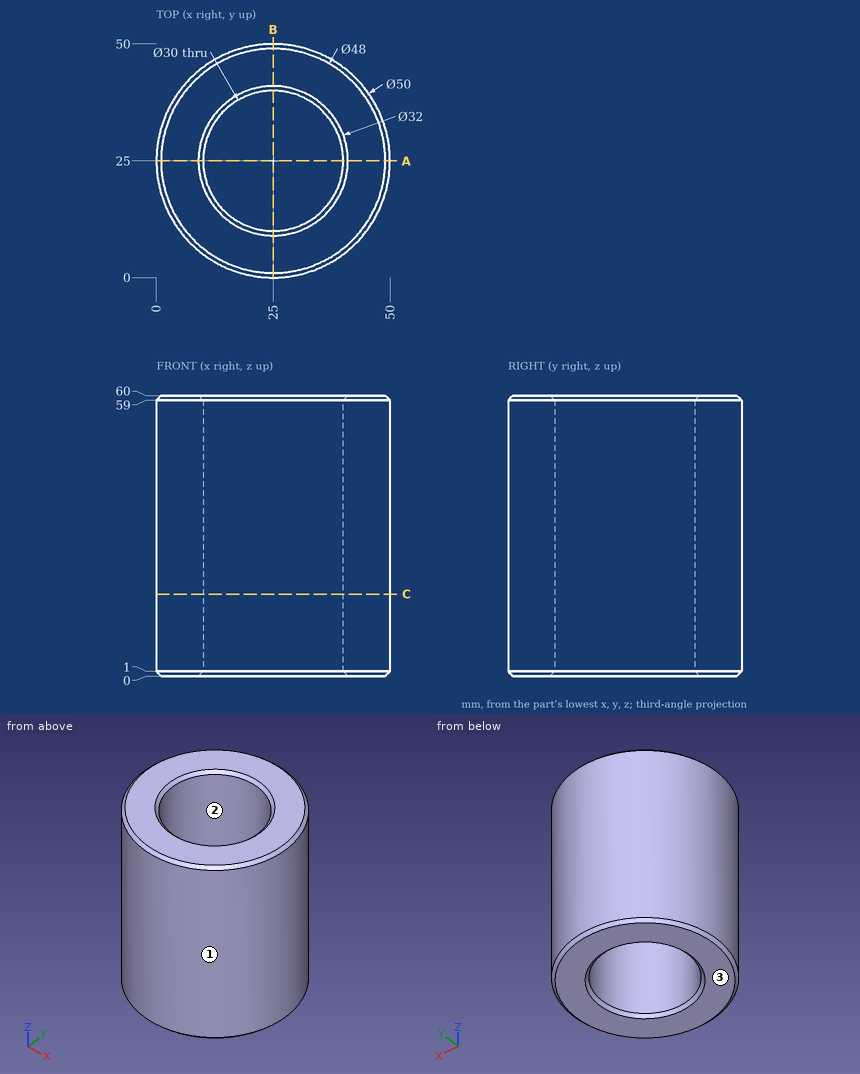
Here's the drawing with two shaded views (mm, measured from the low corner). I have some questions. Round coordinates to 2 decimals unless told otherwise and drop trailing zeros. Loops run counter-clockwise (first coordinate to the right, second up) from the corner with the lowest first, then second, coordinate; pieces in that order, holes last. Notation, with made-up numbers: M -9,5.5 L 23,5.5 A27 cw 23,36.5 Z; hole C 32,39 d8. An arc over 180 degrees is marked long. Answer as a JSON object with one key per item and string values. Group by question number.
Q1. We'd pull the mould along X, two halves only. Please class the marked faces 1, 2 and 3: +X half, -X half, draft (parallel to the pull), parting line (faces both ways), or undercut.
Q2. Imagine slicing it at A-A, the plane y = 25. Please give me the cut outline in (x, z), then the cut area to 3 significant figures.
Q3. Please list where these lines run through material, in increasing order: L1, parallel to Y at x = 25, z = 45.5; L2, parallel to Y at x = 19, z = 54; L3, parallel to X at y = 25.5, z = 20.5 (3 decimals).
Q4. Imagine slicing it at C-C, the plane z = 17.5. Please give me the cut outline in (x, y).
Q5. Will these pins go through, and if not, where does the flat tip stop? pin 1 (4 mm diameter, centred on y = 18, z = 34.5, fed in from -X); pin 2 (5 mm diameter, centred on x = 34.5, y = 38, fed in from -Z); pin 3 (5 mm diameter, centred on x = 26.5, y = 37, fed in from -Z); pin 4 (1.5 mm diameter, centred on x = 29.5, y = 11, fed in from -Z).
Findings:
{
 "1": {"face 1": "parting line", "face 2": "undercut", "face 3": "draft"},
 "2": {"outline": "M 0,1 L 1,0 L 9,0 L 10,1 L 10,59 L 9,60 L 1,60 L 0,59 Z; M 40,1 L 41,0 L 49,0 L 50,1 L 50,59 L 49,60 L 41,60 L 40,59 Z", "area": "1,200 mm2"},
 "3": {"L1": "y = 0 to 10, 40 to 50", "L2": "y = 0.73 to 11.25, 38.75 to 49.27", "L3": "x = 0.005 to 10.008, 39.992 to 49.995"},
 "4": {"outline": "C 25,25 d50; hole C 25,25 d30"},
 "5": {"pin 1": "stops at x = 0.51", "pin 2": "stops at z = 0", "pin 3": "passes through", "pin 4": "stops at z = 0.54"}
}
